from build123d import *

# Parameters (mm, degrees)
SKETCH1_W               = 20
SKETCH1_H               = 17
SKETCH1_W_2             = 18
SKETCH1_H_2             = 3
CUT_EXTRUDE1_DEPTH      = 40.594796465
CUT_EXTRUDE1_DEPTH_BACK = 40.594796465


with BuildPart() as part:
    # Sketch1 → Revolve2 (revolve)
    with BuildSketch(Plane.XY, mode=Mode.PRIVATE) as revolve2_sk:
        with Locations((-10, 9.325484765)):
            Rectangle(SKETCH1_W, SKETCH1_H)
        with Locations((-9, -0.674515235)):
            Rectangle(SKETCH1_W_2, SKETCH1_H_2)
        Polygon((0, -17.174515235), (0, -2.174515235), (-18, -2.174515235), (-25, -2.174515235), (-25, -17.174515235), align=None)
    revolve(revolve2_sk.sketch.rotate(Axis((0, 13.711911357, 0), (0, -1, 0)), 270), axis=Axis((0, 13.711911357, 0), (0, -1, 0)))

    # Sketch3 → Cut-Extrude1 (cut, two sides: drawn at the far end of the back side and taken through both)
    with BuildSketch(Plane.XY.offset(-CUT_EXTRUDE1_DEPTH_BACK)):
        Polygon((-25, -2.174515235), (0, -17.174515235), (-25, -17.174515235), align=None)
    extrude(amount=CUT_EXTRUDE1_DEPTH + CUT_EXTRUDE1_DEPTH_BACK, mode=Mode.SUBTRACT)


solid = part.part
Design review of the part built by this model. Coordinates are the model's own, in mm. A direction names the side the tool comes from. Round coordinates to 2 decimals unless told otherwise and drop trailing zeros. Write each loop counter-clockwise with the first axis right and the second up, starting at its lowest first coordinate (ties: lowest second). Pieces come first, ordered by that corner, then holes. Notation, with made-up numbers: (40, 7.5) - (97, 7.5) arc R29 cw to (97, 36.5) - close; hole circle Ø1 at (-8, -18). An arc over 180 degrees is marked (long way). Use a Markdown table: item, result. Add a question column.
1. We need section B-B (y = 8.5). State the section outline as (x, z) points.
2. Clearance check with flat-ended pins moving along their axes: pin 1 (1.5 mm diameter, centred on x = -2, z = -1, fed in from -Y); pin 2 (5 mm diameter, centred on x = 9.5, y = -6.5, fed in from +Z); pin 3 (5 mm diameter, centred on x = 2.5, y = 11.5, fed in from -Z). State where each tip first meets the part, or that it passes through.
3. For faces 1 (the face through (24.406, -9.78, -5.42)), 2 (the face through (16, -2.175, -11)), list the 3-axis set-ups (+Z, -Z, +X, -X, +Y, -Y) from which the entire face can be reached by the end or side of a thin tool; tool diameter is ignored.
4. We need section A-A (z = 8). State the section outline as (x, y) points.
5. Wall thickness on probe 1 along Y at (x, z) = (22, 4.5); probe 2 along Z at (x, y) = (0.5, -7.5) (3 decimals); probe 3 along X at (y, z) = (6.5, 8.5): over which ranges is each line inside the solid? List them lowest first.
6. We need section D-D (z = 14). State the section outline as (x, y) points.
7. We need section C-C (x = -22). State the section outline as (y, z) points.
8. Mouldability with a two-part tool opening along Y and no side actions: class faces 3 (the face through (-9.897, -11.236, -0.35)), 4 (the face through (-5.407, -0.654, 17.169)), 5 (the face through (19.524, 9.444, -4.336)) as +Y half, -Y half, draft (parallel to the pull), parting line (faces both ways), or undercut.
Output:
| question | item | result |
|---|---|---|
| 1 | outline | circle Ø40 at (0, 0) |
| 2 | pin 1 | stops at y = -16.42 |
| 2 | pin 2 | stops at z = 24 |
| 2 | pin 3 | stops at z = -20 |
| 3 | face 1 | +Y, -Y |
| 3 | face 2 | none |
| 4 | outline | (-23.69, -2.96) - (0, -17.17) - (23.69, -17.17) - (23.69, -2.17) - (16.12, -2.17) - (16.12, 0.83) - (18.33, 0.83) - (18.33, 17.83) - (-18.33, 17.83) - (-18.33, 0.83) - (-16.12, 0.83) - (-16.12, -2.17) - (-23.69, -2.17) - close |
| 5 | probe 1 | y = -17.17 to -2.17 |
| 5 | probe 2 | z = -24.995 to 24.995 |
| 5 | probe 3 | x = -18.1 to 18.1 |
| 6 | outline | (-20.71, -4.75) - (0, -17.17) - (20.71, -17.17) - (20.71, -2.17) - (11.31, -2.17) - (11.31, 0.83) - (14.28, 0.83) - (14.28, 17.83) - (-14.28, 17.83) - (-14.28, 0.83) - (-11.31, 0.83) - (-11.31, -2.17) - (-20.71, -2.17) - close |
| 7 | outline | (-3.97, -11.87) - (-2.17, -11.87) - (-2.17, 11.87) - (-3.97, 11.87) - close |
| 8 | face 3 | -Y half |
| 8 | face 4 | undercut |
| 8 | face 5 | draft |
